```python
from build123d import *


with BuildPart() as part:
    # 草图1 → 旋转1 (revolve)
    with BuildSketch(Plane.XY, mode=Mode.PRIVATE) as revolve_1_sk:
        Polygon((0, 0), (5, 0), (5, 9.5), (6, 9.5), (6, 12.5), (5.5, 12.5), (5.5, 32.5), (10, 32.5), (10, 35.5), (5.5, 35.5), (5.5, 48.5), (10, 48.5), (10, 54.5), (5, 54.5), (5, 67.5), (0, 67.5), align=None)
    revolve(revolve_1_sk.sketch.rotate(Axis((0, -28.718438831, 0), (0, 1, 0)), 90), axis=Axis((0, -28.718438831, 0), (0, 1, 0)))


solid = part.part
```
CAD build for the part. Positions are in the model's coordinates, mm. A direction names the side the tool comes from. Round coordinates to 2 decimals unless told otherwise and drop trailing zeros. Loops run counter-clockwise (first coordinate to the right, second up) from the corner with the lowest first, then second, coordinate; pieces in that order, holes last. Notation, with made-up numbers: M -19,84 L 27,84 A16 ccw 27,108 Z; hole C 41,68.25 d1. An arc over 180 degrees is marked long. Return JSON: item names as keys, results as strings. Group by question number.
(1) Saw through at A-A, the plane x = 0. List the corners of the cut face in (y, z), and give its area (3 significant figures).
(2) Drop flat-ended pins along their axis: P1, Ø10, axis at y = 41.5, z = 1.5, coming from the -X side; P2, Ø3, axis at y = 44.5, z = -4, coming from the +X side; P3, Ø1, axis at y = 18, z = 3.5, coming from the -X side; P4, Ø1.5, axis at y = 10, z = -7, coming from the +X side. Give the stop position or say it passes through.
(3) Saw through at B-B, the plane z = 0. List the corners of the cut face in (x, y).
(4) Wall check: probe 1 along Y at (x, z) = (6.25, 6.5); probe 2 along X at (y, z) = (33, 0.5); probe 3 along X at (y, z) = (16.5, 2.5). Give the ranges that are in metal, low to high. Write a range as [from, to].
(5) Mould opens along Y. For faces 1 (the flat face through (-5, 54.5, -2)), 2 (the flat face through (4, 48.5, 4)), 3 (the flat face through (0, 0, 0)) say: +Y half, -Y half, draft (parallel to the pull), parting line (faces both ways), or undercut.
(6) Tool access for faces 4 (the cylindrical face through (0, 61, 5)), 5 (the cylindrical face through (5.37, 42.09, 1.19)), 6 (the cylindrical face through (0, 5, 5)): list every direction of +Z, -Z, +X, -X, +Y, -Y with a clear straight run to the whole face (end or side of a thin tool).
(7) Saw through at C-C, the plane x = 7.5. List the corners of the cut face in (y, z), and give its area (3 significant figures).
(8) Saw through at D-D, the plane y = 47. List the corners of the cut face in (x, z).
Answer list:
{
 "1": {"outline": "M 0,-5 L 9.5,-5 L 9.5,-6 L 12.5,-6 L 12.5,-5.5 L 32.5,-5.5 L 32.5,-10 L 35.5,-10 L 35.5,-5.5 L 48.5,-5.5 L 48.5,-10 L 54.5,-10 L 54.5,-5 L 67.5,-5 L 67.5,5 L 54.5,5 L 54.5,10 L 48.5,10 L 48.5,5.5 L 35.5,5.5 L 35.5,10 L 32.5,10 L 32.5,5.5 L 12.5,5.5 L 12.5,6 L 9.5,6 L 9.5,5 L 0,5 Z", "area": "804 mm2"},
 "2": {"P1": "x = -5.5", "P2": "x = 4.9", "P3": "x = -4.61", "P4": "through"},
 "3": {"outline": "M -10,32.5 L -5.5,32.5 L -5.5,12.5 L -6,12.5 L -6,9.5 L -5,9.5 L -5,0 L 5,0 L 5,9.5 L 6,9.5 L 6,12.5 L 5.5,12.5 L 5.5,32.5 L 10,32.5 L 10,35.5 L 5.5,35.5 L 5.5,48.5 L 10,48.5 L 10,54.5 L 5,54.5 L 5,67.5 L -5,67.5 L -5,54.5 L -10,54.5 L -10,48.5 L -5.5,48.5 L -5.5,35.5 L -10,35.5 Z"},
 "4": {"probe 1": "[32.5, 35.5], [48.5, 54.5]", "probe 2": "[-9.99, 9.99]", "probe 3": "[-4.9, 4.9]"},
 "5": {"face 1": "+Y half", "face 2": "undercut", "face 3": "-Y half"},
 "6": {"face 4": "+Y", "face 5": "none", "face 6": "-Y"},
 "7": {"outline": "M 32.5,-6.61 L 35.5,-6.61 L 35.5,6.61 L 32.5,6.61 Z; M 48.5,-6.61 L 54.5,-6.61 L 54.5,6.61 L 48.5,6.61 Z", "area": "119 mm2"},
 "8": {"outline": "C 0,0 d11"}
}
